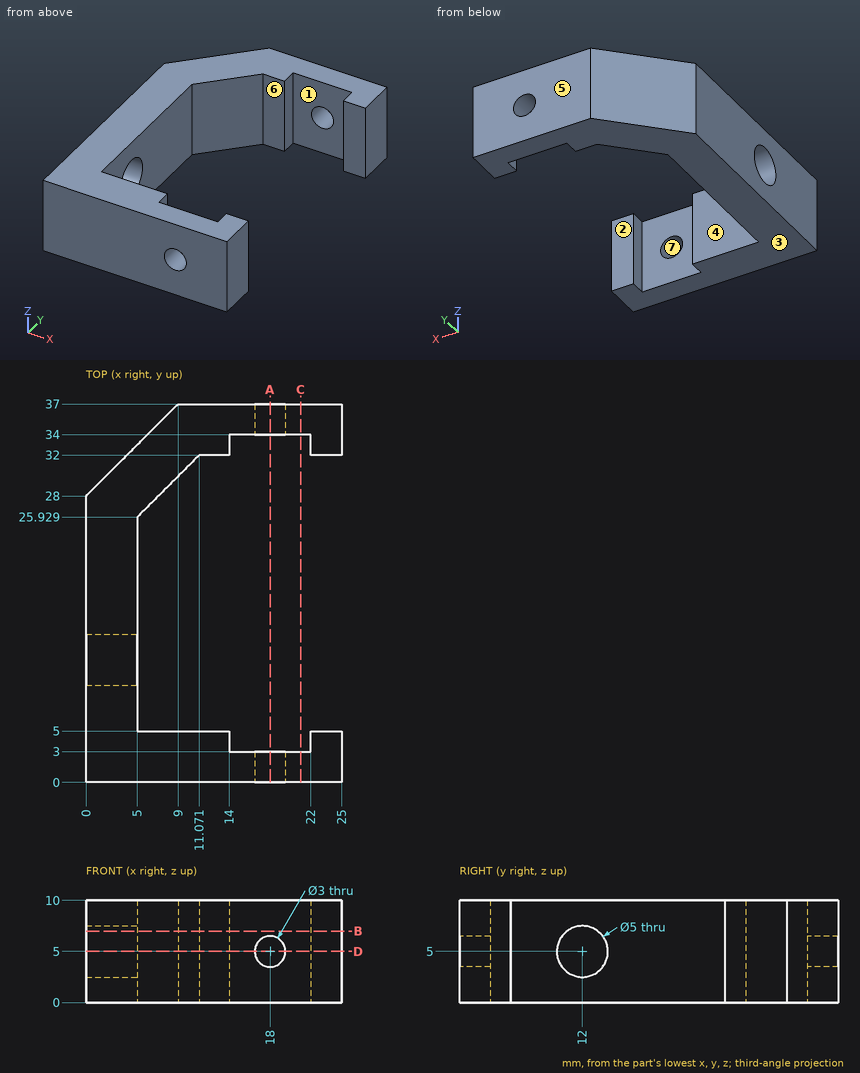
Input: dimensioned drawing with shaded views. Units: mm. Origin: part minimum x, y, z. A direction names the side the tool comes from. Coordinates: 2 decimals unless noted, no trailing zeros. Order: outer loops, then holes, each group sorted by start corner. A loop starts at its lowest first (then second) coordinate and runs counter-clockwise, first axis right, second up. Notation, with made-up numbers: (2.5, -14) - (21.5, -14) arc R5 cw to (21.5, -6) - close; hole circle Ø11 at (35, 36). An arc over 180 degrees is marked (long way). Return JSON: item names as keys, results as strings. Group by question number.
1. Pull-direction query (Y, two-part tool) for the marked faces 4, 5, 6 and 7; classes: pulls with the +Y half, pulls with the -Y half, needs draft (parallel to the pull), parting line crosses it, or undercut.
2. Cut plane D-D (z = 5). Count the separate pieces of the cut face and the enclosed holes in it, plus the area to 3 significant figures.
3. Set-up query: the marked faces 1, 2 and 3. Return all of +Z, -Z, +X, -X, +Y, -Y with unobstructed straight access to the full face (end or side cutting, diameter ignored); none if empty.
4. Material intervals for line 1 along Y through (x, z) = (19.5, 6.25); line 2 along X through (y, z) = (1.95, 5); line 3 along Y through (x, z) = (11.25, 2.75), sorted ascending. Write a range as [from, to].
5. Cut plane C-C (x = 21). Output: boundary loops of the cut face in (y, z), plus the area to 3 significant figures.
6. Cut plane B-B (z = 7). Output: boundary loops of the cut face in (x, y), plus the area to 3 significant figures.
7. Cut plane A-A (x = 18). Output: boundary loops of the cut face in (y, z), plus the area to 3 significant figures.
8. Pin query (flat end, axial travel): pin 1 (0.6 mm diameter, centred on y = 32.5, z = 6, fed in from -X). Return the tip coordinate at first contact, or that it passes through.
Resolved:
{
 "1": {"face 4": "undercut", "face 5": "pulls with the +Y half", "face 6": "undercut", "face 7": "needs draft"},
 "2": {"separate pieces": "4", "enclosed holes": "0", "area": "288 mm²"},
 "3": {"face 1": "+Z, -Z", "face 2": "+Z, -Z, +X", "face 3": "-Z, +X, -X, +Y, -Y"},
 "4": {"line 1": "y = [0, 3], [34, 37]", "line 2": "x = [0, 16.5], [19.5, 25]", "line 3": "y = [0, 5], [32, 37]"},
 "5": {"outline": "(0, 0) - (3, 0) - (3, 10) - (0, 10) - close; (34, 0) - (37, 0) - (37, 10) - (34, 10) - close", "area": "60.0 mm²"},
 "6": {"outline": "(0, 0) - (25, 0) - (25, 5) - (22, 5) - (22, 3) - (14, 3) - (14, 5) - (5, 5) - (5, 10.5) - (0, 10.5) - close; (0, 13.5) - (5, 13.5) - (5, 25.93) - (11.07, 32) - (14, 32) - (14, 34) - (22, 34) - (22, 32) - (25, 32) - (25, 37) - (9, 37) - (0, 28) - close", "area": "316 mm²"},
 "7": {"outline": "(0, 0) - (3, 0) - (3, 3.5) - (0, 3.5) - close; (0, 6.5) - (3, 6.5) - (3, 10) - (0, 10) - close; (34, 0) - (37, 0) - (37, 3.5) - (34, 3.5) - close; (34, 6.5) - (37, 6.5) - (37, 10) - (34, 10) - close", "area": "42.0 mm²"},
 "8": {"pin 1": "stops at x = 4.2"}
}
